from build123d import *

# Parameters (mm, degrees)
SKETCH_1_W                  = 200
SKETCH_1_H                  = 270
EXTRUDE_1_DEPTH             = 12
SKETCH_2_W                  = 121
SKETCH_2_H                  = 270
CUT_EXTRUDE_1_DEPTH         = 3
CHAMFER_1_SIZE              = 5
CHAMFER_1_SIZE2             = 8.660254038
HOLE_WIZARD_M5_1_AT_2_COUNT = 2
HOLE_WIZARD_M5_1_AT_2_PITCH = 180
CHAMFER_2_SIZE              = 1
MM_1_D                      = 5


with BuildPart() as part:
    # 草图1 → 凸台-拉伸1 (new body)
    with BuildSketch(Plane.XY):
        Rectangle(SKETCH_1_W, SKETCH_1_H)
    extrude(amount=EXTRUDE_1_DEPTH)

    # 草图2 → 切除-拉伸1 (cut)
    with BuildSketch(Plane.XY.offset(12)):
        with Locations((-1, 0)):
            Rectangle(SKETCH_2_W, SKETCH_2_H)
    extrude(amount=-CUT_EXTRUDE_1_DEPTH, mode=Mode.SUBTRACT)

    # 倒角1
    chamfer_1_edges = [part.edges().sort_by_distance(p)[0] for p in [
        (59.5, 135, 10.5),
        (-61.5, 135, 10.5),
    ]]
    chamfer_1_side = [part.faces().sort_by_distance(p)[0] for p in [
        (0.17820324, 135, 5.19808542),
    ]]
    chamfer(chamfer_1_edges, length=CHAMFER_1_SIZE, length2=CHAMFER_1_SIZE2, reference=chamfer_1_side[0])

    # 草图4 → M5 螺纹孔1 (revolve, cut)
    with BuildSketch(Plane(origin=(90, 135, 6), x_dir=(0, 0, 1), z_dir=(1, 0, 0))):
        Polygon((0, 0), (0, 13.6618073), (2.1, 12.4), (2.1, 0), align=None)
    hole_wizard_m5_1 = revolve(axis=Axis((90, 141.35, 6), (0, -1, 0)), mode=Mode.SUBTRACT)

    # M5 螺纹孔1 at 2: M5 螺纹孔1 ×2
    with Locations(*[(-i * HOLE_WIZARD_M5_1_AT_2_PITCH, 0, 0) for i in range(1, HOLE_WIZARD_M5_1_AT_2_COUNT)]):
        add(hole_wizard_m5_1, mode=Mode.SUBTRACT)

    # 镜向1: M5 螺纹孔1 across plane
    add(hole_wizard_m5_1.mirror(Plane.ZX), mode=Mode.SUBTRACT)

    # 镜向1 copy 1 sketch → 镜向1 copy 1 (revolve, cut)
    with BuildSketch(Plane(origin=(-90, -135, 6), x_dir=(0, 0, 1), z_dir=(1, 0, 0))):
        Polygon((0, 0), (0, -13.6618073), (2.1, -12.4), (2.1, 0), align=None)
    revolve(axis=Axis((-90, -141.35, 6), (0, -1, 0)), mode=Mode.SUBTRACT)

    # 倒角2
    chamfer_2_edges = [part.edges().sort_by_distance(p)[0] for p in [
        (-100, 0, 12),
        (-80.75, -135, 12),
        (79.75, -135, 12),
        (-83.25, 135, 12),
        (100, 0, 12),
        (0, -135, 0),
        (-100, 0, 0),
        (0, 135, 0),
        (100, 0, 0),
        (82.25, 135, 12),
        (100, -135, 6),
        (-100, -135, 6),
        (-100, 135, 6),
        (100, 135, 6),
    ]]
    chamfer(chamfer_2_edges, length=CHAMFER_2_SIZE)

    # 大小mm 暗销孔1 (through all)
    with Locations(Plane.XY.offset(9)):
        with Locations((-1, -87.5)):
            Hole(MM_1_D / 2)


solid = part.part
Input: part model. Units: mm. Frame: model coordinates. Give positions to 0.01 mm unless a question says otherwise; leave off trailing zeros. Order: outer loops, then holes, each group sorted by start corner. A loop starts at its lowest first (then second) coordinate and runs counter-clockwise, first axis right, second up. Notation, with made-up numbers: (17, -4.75) -> (30, -4.75) arc R20 ccw to (30, 29.25) -> close; hole circle Ø1 at (8.25, 18.5). An arc over 180 degrees is marked (long way). Use one line per item in the form item = value.
1) Line query: probe 1 along X at (y, z) = (128.75, 6); probe 2 along Z at (x, y) = (-90, -130); probe 3 along X at (y, z) = (-84, 11). Output: solid intervals per line, ascending.
Response values:
probe_1 = -100 to -92.1, -87.9 to 87.9, 92.1 to 100
probe_2 = 0 to 3.9, 8.1 to 12
probe_3 = -100 to -61.5, 59.5 to 100
2) Section A-A, the plane y = 85. Return loops of the section in (x, z), and give its area (4 significant figures).
Response values:
outline = (-100, 1) -> (-99, 0) -> (99, 0) -> (100, 1) -> (100, 11) -> (99, 12) -> (59.5, 12) -> (59.5, 9) -> (-61.5, 9) -> (-61.5, 12) -> (-99, 12) -> (-100, 11) -> close
area = 2,035 mm^2
3) Section B-B, the plane x = -51. Return loops of the section in (y, z), and give its area (3 significant figures).
Response values:
outline = (-135, 1) -> (-134, 0) -> (134, 0) -> (135, 1) -> (135, 9) -> (-135, 9) -> close
area = 2,430 mm^2
4) First-contact query: pin 1 Ø2.5 at (x, z) = (90, 6) entering from -Y; pin 2 Ø2.5 at (x, z) = (90, 6) entering from +Y. Flat tips, straight axial feed; report the tip coordinate or a pass-through.
Response values:
pin_1 = -122.09
pin_2 = 122.09
5) Mould query, pull axis X, two halves, no side actions, for faces 1 (the flat face through (100, -2, 6)), 2 (the flat face through (79, 2, 12)), 3 (the flat face through (-2, 2, 9)). Classes: pulls with the +X half, pulls with the -X half, needs draft (parallel to the pull), parting line crosses it, or undercut.
Response values:
face_1 = pulls with the +X half
face_2 = needs draft
face_3 = undercut
